from build123d import *

# Parameters (mm, degrees)
SKETCH1_W                                         = 185
SKETCH1_H                                         = 50
BOSS_EXTRUDE1_DEPTH                               = 25
SKETCH2_W                                         = 62.5
SKETCH2_H                                         = 50
CUT_EXTRUDE1_DEPTH                                = 11.5
M5_SOCKET_HEAD_CAP_SCREW_COUNTERBORE1_D           = 5.5
M5_SOCKET_HEAD_CAP_SCREW_COUNTERBORE1_CBORE_D     = 10
M5_SOCKET_HEAD_CAP_SCREW_COUNTERBORE1_CBORE_DEPTH = 5.7
M5_SOCKET_HEAD_CAP_SCREW_COUNTERBORE2_D           = 5.5
M5_SOCKET_HEAD_CAP_SCREW_COUNTERBORE2_CBORE_D     = 10
M5_SOCKET_HEAD_CAP_SCREW_COUNTERBORE2_CBORE_DEPTH = 5.7


with BuildPart() as part:
    # Sketch1 → Boss-Extrude1 (new body)
    with BuildSketch(Plane.XY):
        Rectangle(SKETCH1_W, SKETCH1_H)
    extrude(amount=BOSS_EXTRUDE1_DEPTH)

    # Sketch2 → Cut-Extrude1 (cut)
    with BuildSketch(Plane.XY.offset(25)):
        with Locations((-61.25, 0)):
            Rectangle(SKETCH2_W, SKETCH2_H)
        with Locations((61.25, 0)):
            Rectangle(SKETCH2_W, SKETCH2_H)
    extrude(amount=-CUT_EXTRUDE1_DEPTH, mode=Mode.SUBTRACT)

    # M5 socket head cap screw counterbore1 (through all)
    with Locations(Plane(origin=(0, 0, 0), x_dir=(-1, 0, 0), z_dir=(0, 0, -1))):
        with Locations((-86, 0), (-60, 0), (60, 0), (86, 0)):
            CounterBoreHole(M5_SOCKET_HEAD_CAP_SCREW_COUNTERBORE1_D / 2, M5_SOCKET_HEAD_CAP_SCREW_COUNTERBORE1_CBORE_D / 2, M5_SOCKET_HEAD_CAP_SCREW_COUNTERBORE1_CBORE_DEPTH)

    # M5 socket head cap screw counterbore2 (through all)
    with Locations(Plane(origin=(0, 0, 0), x_dir=(-1, 0, 0), z_dir=(0, 0, -1))):
        with Locations((-22.5, 12.5), (-22.5, -12.5), (22.5, 12.5), (22.5, -12.5)):
            CounterBoreHole(M5_SOCKET_HEAD_CAP_SCREW_COUNTERBORE2_D / 2, M5_SOCKET_HEAD_CAP_SCREW_COUNTERBORE2_CBORE_D / 2, M5_SOCKET_HEAD_CAP_SCREW_COUNTERBORE2_CBORE_DEPTH)


solid = part.part
Verification items for the finished model (mm, model axes). A direction names the side the tool comes from. Round coordinates to 2 decimals unless told otherwise and drop trailing zeros. Write each loop counter-clockwise with the first axis right and the second up, starting at its lowest first coordinate (ties: lowest second). Pieces come first, ordered by that corner, then holes.
(1) Mould release check, pull along X, two halves, no side actions. Record for faces 4 (the flat face through (61, 6, 13.5)), 5 (the flat face through (92.5, 0, 7)), 6 (the cylindrical face through (-25.247, 12.621, 15.485)): pulls with the +X half, pulls with the -X half, needs draft (parallel to the pull), parting line crosses it, or undercut.
Returned:
face 4: needs draft
face 5: pulls with the +X half
face 6: undercut
(2) Section check B-B (z = 17.75). Enter the section's corners in (x, y).
Returned:
outline: (-30, -25) - (30, -25) - (30, 25) - (-30, 25) - close; hole circle Ø5.5 at (-22.5, -12.5); hole circle Ø5.5 at (-22.5, 12.5); hole circle Ø5.5 at (22.5, -12.5); hole circle Ø5.5 at (22.5, 12.5)
(3) Material ranges on line 1 (Y direction, x = 22.5, z = 17.75); line 2 (Y direction, x = -22.5, z = 1.3); line 3 (Y direction, x = 60, z = 12.25), recorded low to high.
Returned:
line 1: y = -25 to -15.25, -9.75 to 9.75, 15.25 to 25
line 2: y = -25 to -17.5, -7.5 to 7.5, 17.5 to 25
line 3: y = -25 to -2.75, 2.75 to 25
(4) Section check A-A (x = 22.5). Enter the section's corners in (y, z).
Returned:
outline: (-25, 0) - (-17.5, 0) - (-17.5, 5.7) - (-15.25, 5.7) - (-15.25, 25) - (-25, 25) - close; (-9.75, 5.7) - (-7.5, 5.7) - (-7.5, 0) - (7.5, 0) - (7.5, 5.7) - (9.75, 5.7) - (9.75, 25) - (-9.75, 25) - close; (15.25, 5.7) - (17.5, 5.7) - (17.5, 0) - (25, 0) - (25, 25) - (15.25, 25) - close
(5) Section check D-D (y = 12.5). Enter the section's corners in (x, z).
Returned:
outline: (-92.5, 0) - (-27.5, 0) - (-27.5, 5.7) - (-25.25, 5.7) - (-25.25, 25) - (-30, 25) - (-30, 13.5) - (-92.5, 13.5) - close; (-19.75, 5.7) - (-17.5, 5.7) - (-17.5, 0) - (17.5, 0) - (17.5, 5.7) - (19.75, 5.7) - (19.75, 25) - (-19.75, 25) - close; (25.25, 5.7) - (27.5, 5.7) - (27.5, 0) - (92.5, 0) - (92.5, 13.5) - (30, 13.5) - (30, 25) - (25.25, 25) - close
(6) Depth check by flat-ended pin: pin 1 Ø8 at (x, y) = (86, 0) entering from +Z; pin 2 Ø5 at (x, y) = (62, -0.5) entering from -Z; pin 3 Ø3.5 at (x, y) = (-60, 0) entering from +Z. Enter the tip coordinate at first touch or a pass-through.
Returned:
pin 1: stops at z = 13.5
pin 2: stops at z = 5.7
pin 3: passes through
(7) Section check C-C (x = 86). Enter the section's corners in (y, z), plus the area to 3 significant figures.
Returned:
outline: (-25, 0) - (-5, 0) - (-5, 5.7) - (-2.75, 5.7) - (-2.75, 13.5) - (-25, 13.5) - close; (2.75, 5.7) - (5, 5.7) - (5, 0) - (25, 0) - (25, 13.5) - (2.75, 13.5) - close
area: 575 mm2
(8) Access from +Z, -Z, +X, -X, +Y, -Y to the whole of each face (thin tool, end or side, straight path). Record for faces 1 (the flat face through (30, 0, 19)), 2 (the cylindrical face through (-90.619, -1.915, 2.81)), 3 (the flat face through (-30, 0, 19)).
Returned:
face 1: +Z, +X, +Y, -Y
face 2: -Z
face 3: +Z, -X, +Y, -Y
